Model file for the job. Use its own axes, mm. A direction names the side the tool comes from. Coordinates: 2 decimals unless noted, no trailing zeros. Write each loop counter-clockwise with the first axis right and the second up, starting at its lowest first coordinate (ties: lowest second). Pieces come first, ordered by that corner, then holes. Notation, with made-up numbers: M -16,22 L 10,22 A23 cw 10,34 Z; hole C -23.5,59.25 d9. An arc over 180 degrees is marked long. Answer in a Markdown table with one row per item. Add a question column.
```python
from build123d import *

# Parameters (mm, degrees)
EXTRUDE_1_DEPTH        = 100
SKETCH_2_W             = 4
SKETCH_2_H             = 20
EXTRUDE_2_DEPTH        = 100
PATTERN_LINEAR_1_COUNT = 5
PATTERN_LINEAR_1_PITCH = 60
SKETCH_3_W             = 4
SKETCH_3_H             = 20
EXTRUDE_3_DEPTH        = 100
PATTERN_LINEAR_2_COUNT = 5
PATTERN_LINEAR_2_PITCH = 60


with BuildPart() as part:
    # 草图1 → 凸台-拉伸1 (new body)
    with BuildSketch(Plane.XY):
        with BuildLine():
            Line((0, 27), (250, 27))
            ThreePointArc((250, 27), (277, 0), (250, -27))
            Line((250, -27), (0, -27))
            ThreePointArc((0, -27), (-27, 0), (0, 27))
        make_face()
        with BuildLine():
            Line((0, 25), (250, 25))
            ThreePointArc((250, 25), (275, 0), (250, -25))
            Line((250, -25), (0, -25))
            ThreePointArc((0, -25), (-25, 0), (0, 25))
        make_face(mode=Mode.SUBTRACT)
    extrude(amount=EXTRUDE_1_DEPTH)

    # 草图2 → 凸台-拉伸2 (add)
    with BuildSketch(Plane.XY.offset(100)):
        with Locations((2, 37)):
            Rectangle(SKETCH_2_W, SKETCH_2_H)
    extrude_2 = extrude(amount=-EXTRUDE_2_DEPTH)

    # 阵列(线性)1: 凸台-拉伸2 ×5
    with Locations(*[(i * PATTERN_LINEAR_1_PITCH, 0, 0) for i in range(1, PATTERN_LINEAR_1_COUNT)]):
        add(extrude_2)

    # 草图3 → 凸台-拉伸3 (add)
    with BuildSketch(Plane.XY.offset(100)):
        with Locations((2, -37)):
            Rectangle(SKETCH_3_W, SKETCH_3_H)
    extrude_3 = extrude(amount=-EXTRUDE_3_DEPTH)

    # 阵列(线性)2: 凸台-拉伸3 ×5
    with Locations(*[(i * PATTERN_LINEAR_2_PITCH, 0, 0) for i in range(1, PATTERN_LINEAR_2_COUNT)]):
        add(extrude_3)


solid = part.part
```
1) Slice it at B-B (x = 79.5). Give the cut face in (y, z).
2) Slice it at A-A (y = 0). Give the cut face in (x, z).
3) Flat gauge pins, fed straight in: pin 1 Ø16 at (y, z) = (-33, 64.5) entering from -X; pin 2 Ø22 at (y, z) = (32.5, 62.5) entering from -X; pin 3 Ø16 at (y, z) = (-37, 32.5) entering from +X. Where does each tip first touch, or does it go through?
4) Drill centre lines: probe 1 along X at (y, z) = (29, 61); probe 2 along Y at (x, z) = (0.5, 16.5); probe 3 along Y at (x, z) = (175, 37). Where is each one in solid material? Low to high.
5) Which spindle directions (+Z, -Z, +X, -X, +Y, -Y) get a long thin tool onto all of the face, cutting with end or side? Do faces 4 (the face through (-24.994, -0.55, 49.3)), 5 (the face through (124, -37, 51)), 6 (the face through (247, 27, 49)), 7 (the face through (92, 27, 49)). Say none if no direction does.
6) Two-plate mould, pull along X, no slides. Class faces 1 (the face through (181, -28, 0)), 2 (the face through (4, -37, 51)), 3 (the face through (0, -37, 51)): released by +X, released by -X, zero draft, split by the parting line, or undercut.
Ans:
| question | item | result |
|---|---|---|
| 1 | outline | M -27,0 L -25,0 L -25,100 L -27,100 Z; M 25,0 L 27,0 L 27,100 L 25,100 Z |
| 2 | outline | M -27,0 L -25,0 L -25,100 L -27,100 Z; M 275,0 L 277,0 L 277,100 L 275,100 Z |
| 3 | pin 1 | stops at x = -10.2 |
| 3 | pin 2 | stops at x = -16.33 |
| 3 | pin 3 | stops at x = 244 |
| 4 | probe 1 | x = 0 to 4, 60 to 64, 120 to 124, 180 to 184, 240 to 244 |
| 4 | probe 2 | y = -47 to -25, 25 to 47 |
| 4 | probe 3 | y = -27 to -25, 25 to 27 |
| 5 | face 4 | +Z, -Z |
| 5 | face 5 | +Z, -Z, -Y |
| 5 | face 6 | +Z, -Z, +X, +Y |
| 5 | face 7 | +Z, -Z, +Y |
| 6 | face 1 | zero draft |
| 6 | face 2 | undercut |
| 6 | face 3 | released by -X |
